Build history of the part. All positions in model axes, mm. A direction names the side the tool comes from. Round coordinates to 2 decimals unless told otherwise and drop trailing zeros. Write each loop counter-clockwise with the first axis right and the second up, starting at its lowest first coordinate (ties: lowest second). Pieces come first, ordered by that corner, then holes.
Item 1: Band-saw the part on B-B, the plane x = 109.5. Write the cut outline in (y, z), then the cut area to 3 significant figures.
Item 2: Wall check: probe 1 along X at (y, z) = (0.5, -136.5); probe 2 along Y at (x, z) = (500, -130); probe 3 along X at (y, z) = (-8.5, -58). Give the ranges that are in metal, low to high.
Item 3: Drop flat-ended pins along their axis: pin 1 Ø7.5 at (x, y) = (500, 0) entering from +Z; pin 2 Ø6 at (y, z) = (-5, -68.5) entering from +X; pin 3 Ø1.5 at (x, z) = (343.5, -3.5) entering from +Y. Give the stop position or say it passes through.
Item 4: Band-saw the part on A-A, the plane y = 9.5. Write the cut outline in (x, z).
Item 5: 3-axis set-ups, long thin cutter, end or side, ignore diameter. For faces 1 (the cylindrical face through (513.856, -5.745, -124.65)), 2 (the flat face through (-3.12, -3.12, -150)), 3 (the cylindrical face through (247.9, 0.66, -14.985)): which of +Z, -Z, +X, -X, +Y, -Y reach the whole face in a straight line?
Item 6: Mould opens along X. For faces 4 (the conical face through (0.16, -0.72, -116.39)), 5 (the flat face through (503.12, -3.12, -150)), 6 (the conical face through (499.296, 0.222, -116.39)) say: +X half, -X half, draft (parallel to the pull), parting line (faces both ways), or undercut.
```python
from build123d import *

# Parameters (mm, degrees)
SWEEP1_PROFILE_R       = 15
M10_TAPPED_HOLE1_D     = 8.5
M10_TAPPED_HOLE1_DEPTH = 31.5
M10_TAPPED_HOLE1_TIP   = 2.553657631


with BuildPart() as part:
    # Sweep1: sweep along a path in Sketch1
    with BuildLine(Plane(origin=(0, 0, 0), x_dir=(1, 0, 0), z_dir=(0, 1, 0))) as sweep1_path:
        Line((500, 150), (500, 100))
        ThreePointArc((500, 100), (470.710678119, 29.289321881), (400, 0))
        Line((400, 0), (100, 0))
        ThreePointArc((100, 0), (29.289321881, 29.289321881), (0, 100))
        Line((0, 100), (0, 150))
    # Sweep1 profile (on start of the path) → Sweep1 (sweep)
    with BuildSketch(Plane(origin=(500, 0, -150), x_dir=(1, 0, 0), z_dir=(0, 0, 1))):
        Circle(SWEEP1_PROFILE_R)
    sweep(path=sweep1_path.line)

    # M10 Tapped Hole1
    with Locations(Plane(origin=(0, 0, -150), x_dir=(-1, 0, 0), z_dir=(0, 0, -1))):
        with Locations((-500, 0), (0, 0)):
            Hole(M10_TAPPED_HOLE1_D / 2, depth=M10_TAPPED_HOLE1_DEPTH)
            with Locations((0, 0, -(M10_TAPPED_HOLE1_DEPTH + M10_TAPPED_HOLE1_TIP / 2))):  # 118° drill point
                Cone(0, M10_TAPPED_HOLE1_D / 2, M10_TAPPED_HOLE1_TIP, mode=Mode.SUBTRACT)


solid = part.part
```
Results:
1. outline: circle Ø30 at (0, 0)
1. area: 707 mm2
2. probe 1: x = -14.99 to -4.22, 4.22 to 14.99, 485.01 to 495.78, 504.22 to 514.99
2. probe 2: y = -15 to -4.25, 4.25 to 15
2. probe 3: x = -4.21 to 23.08, 476.92 to 504.21
3. pin 1: stops at z = -37.06
3. pin 2: stops at x = 510.9
3. pin 3: stops at y = 14.75
4. outline: (-11.61, -150) - (11.61, -150) - (11.61, -100) arc R88.39 cw to (100, -11.61) - (400, -11.61) arc R88.39 cw to (488.39, -100) - (488.39, -150) - (511.61, -150) - (511.61, -100) arc R111.61 ccw to (400, 11.61) - (100, 11.61) arc R111.61 ccw to (-11.61, -100) - close
5. face 1: -Z
5. face 2: -Z, +X, -X, +Y, -Y
5. face 3: none
6. face 4: undercut
6. face 5: draft
6. face 6: undercut
